Can you work these out from the model? Positions are in its coordinate system, mm. Face numbers are marked on the shaded views. A direction names the side the tool comes from. Give positions to 0.01 mm unless a question says otherwise; leave off trailing zeros. Loops run counter-clockwise (first coordinate to the right, second up) from the corner with the lowest first, then second, coordinate; pieces in that order, holes last. Notation, with made-up numbers: M 15.5,28.5 L 46.5,28.5 A25 ccw 46.5,60.5 Z; hole C 38.5,65 d10. An arc over 180 degrees is marked long. One line per item, written item: value. Start each with the question number.
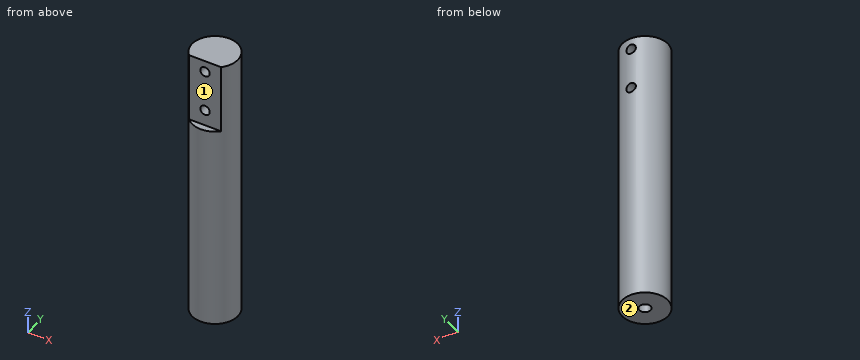
from build123d import *

# Parameters (mm, degrees)
SKETCH_1_R             = 10
EXTRUDE_1_DEPTH        = 60
HOLE_WIZARD_M6_1_D     = 5
HOLE_WIZARD_M6_1_DEPTH = 15
HOLE_WIZARD_M6_1_TIP   = 1.502151548
SKETCH_5_W             = 14.282856858
SKETCH_5_H             = 6
CUT_EXTRUDE_1_DEPTH    = 30
HOLE_WIZARD_M5_1_D     = 4.2


with BuildPart() as part:
    # 草图1 → 凸台-拉伸1 (new, symmetric)
    with BuildSketch(Plane.XY):
        Circle(SKETCH_1_R)
    extrude(amount=EXTRUDE_1_DEPTH, both=True)

    # M6 螺纹孔1
    with Locations(Plane(origin=(0, 0, -60), x_dir=(-1, 0, 0), z_dir=(0, 0, -1))):
        with Locations((0, 0)):
            Hole(HOLE_WIZARD_M6_1_D / 2, depth=HOLE_WIZARD_M6_1_DEPTH)
            with Locations((0, 0, -(HOLE_WIZARD_M6_1_DEPTH + HOLE_WIZARD_M6_1_TIP / 2))):  # 118° drill point
                Cone(0, HOLE_WIZARD_M6_1_D / 2, HOLE_WIZARD_M6_1_TIP, mode=Mode.SUBTRACT)

    # 草图5 → 切除-拉伸1 (cut)
    with BuildSketch(Plane.XY.offset(60)):
        with Locations((0, -10)):
            Rectangle(SKETCH_5_W, SKETCH_5_H)
    extrude(amount=-CUT_EXTRUDE_1_DEPTH, mode=Mode.SUBTRACT)

    # M5 螺纹孔1 (through all)
    with Locations(Plane(origin=(0, -7, 0), x_dir=(-1, 0, 0), z_dir=(0, -1, 0))):
        with Locations((0, -55), (0, -37)):
            Hole(HOLE_WIZARD_M5_1_D / 2)


solid = part.part
Q1. If we section it at D-D, the plane z = 5.5: Write out the boundary of the cut face in (x, y), plus the area to 3 significant figures.
Q2. I need wall thicknesses on line 1 along Z through (x, y) = (0, 4.5); line 2 along Z through (x, y) = (0, 0); line 3 along X through (y, z) = (0, -55.5). Which ranges of each line are inside material? Lowest first, please.
Q3. If we section it at B-B, the plane z = 46: Write out the boundary of the cut face in (x, y).
Q4. Which directions (+Z, -Z, +X, -X, +Y, -Y) give clear straight access to the entire face, cutting with the end or side of a thin tool? Please do the marked faces 1 and 2.
Q5. If we section it at A-A, the plane y = 7: Write out the boundary of the cut face in (x, z).
Q6. For P1, Ø2, axis at y = 2.5, z = 32.5, coming from the -X side; P2, Ø3, axis at x = 6, z = 4.5, coming from the +Y side; P3, Ø4, axis at x = -3.5, z = -21, coming from the -Y side; P4, Ø6, axis at x = 0, y = 0, coming from the -Z side, each with a flat end and sliding along its axis, tell me the tip position at first contact or that it passes through.
Q7. If we section it at C-C, the plane x = 5.75: Write out the boundary of the cut face in (y, z), plus the area to 3 significant figures.
Response:
1. outline: C 0,0 d20
1. area: 314 mm^2
2. line 1: -60 to 34.9, 39.1 to 52.9, 57.1 to 60
2. line 2: -43.5 to 34.9, 39.1 to 52.9, 57.1 to 60
2. line 3: -10 to -2.5, 2.5 to 10
3. outline: M -7.14,-7 L 7.14,-7 A10 ccw long Z
4. face 1: +Z, +X, -X, -Y
4. face 2: -Z, +X, -X, +Y, -Y
5. outline: M -7.14,-60 L 7.14,-60 L 7.14,60 L -7.14,60 Z; hole C 0,37 d4.2; hole C 0,55 d4.2
6. P1: x = -9.89
6. P2: y = 8.93
6. P3: y = -9.89
6. P4: z = -60
7. outline: M -8.18,-60 L 8.18,-60 L 8.18,60 L -7,60 L -7,30 L -8.18,30 Z
7. area: 1,930 mm^2
